Geometry: see drawing. Coordinates: mm, zero at the bounding-box minimum. A direction names the side the tool comes from. Give positions to 0.01 mm unless a question says otherwise; leave off trailing zeros. Loops run counter-clockwise (first coordinate to the right, second up) from the corner with the lowest first, then second, coordinate; pieces in that order, holes last. Notation, with made-up numbers: (39.5, 75) -> (77.5, 75) arc R30 cw to (77.5, 110) -> close; hole circle Ø3 at (-19.75, -7). An arc over 180 degrees is marked (long way). Answer in a Markdown table with one row per item. Add a question column.
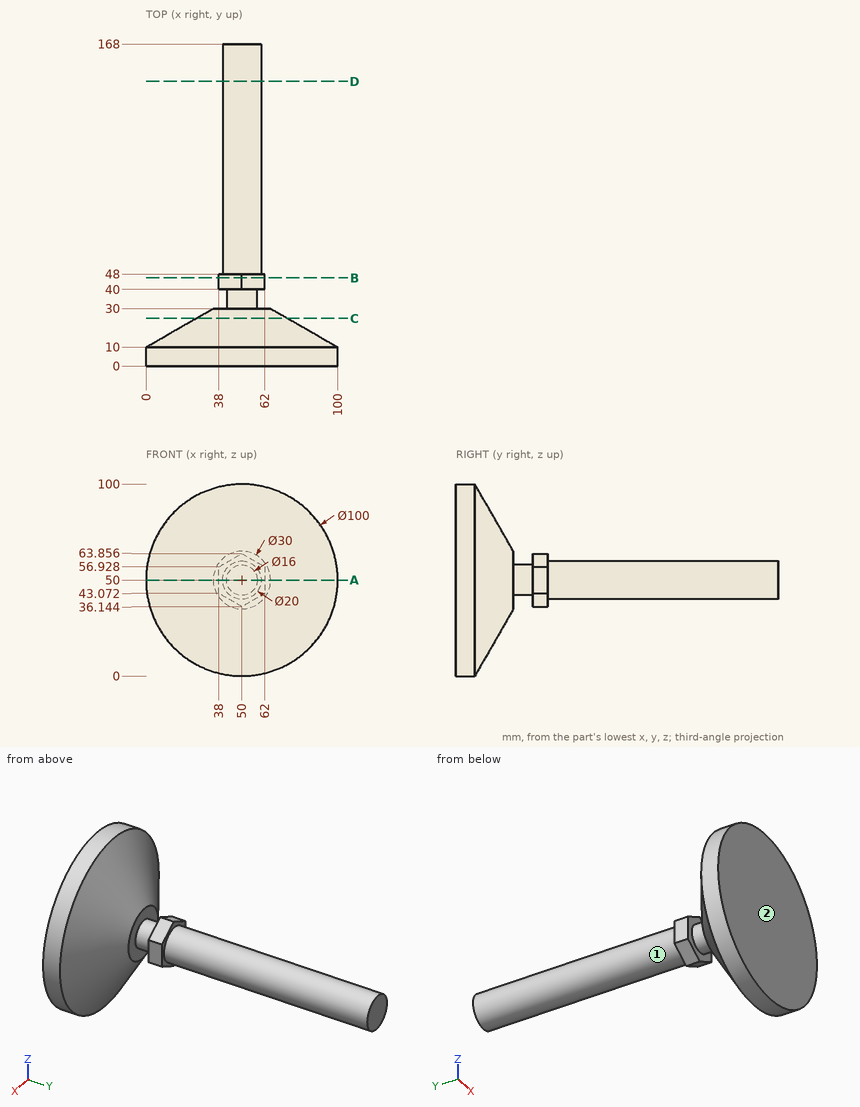
1) Section B-B on y = 46. Output: boundary loops of the cut face in (x, z), and give its area (3 significant figures).
2) Section C-C on y = 25. Output: boundary loops of the cut face in (x, z).
3) Section D-D on y = 148.5. Output: boundary loops of the cut face in (x, z).
4) Reachability of the marked faces 1 and 2 from +Z, -Z, +X, -X, +Y, -Y: full face, straight path, thin tool, end or side. Return the list, or none.
5) Section A-A on z = 50. Output: boundary loops of the cut face in (x, y).
6) Material intervals for line 1 along X through (y, z) = (21, 69) (1 decimal); line 2 along Y through (x, z) = (33, 47); line 3 along Y through (x, z) = (66, 66), sorted ascending.
7) Pin query (flat end, axial travel): pin 1 (12 mm diameter, centred on y = 61.5, z = 41.5, fed in from -X); pin 2 (6 mm diameter, centred on y = 131.5, z = 42, fed in from -X); pin 3 (6.5 mm diameter, centred on y = 42.5, z = 48, fed in from +X); pin 4 (1 mm diameter, centred on x = 38.5, y = 130, fed in from +Z). Return the tip coordinate at first contact, or that it passes through.
Working result:
| question | item | result |
|---|---|---|
| 1 | outline | (38, 43.07) -> (50, 36.14) -> (62, 43.07) -> (62, 56.93) -> (50, 63.86) -> (38, 56.93) -> close |
| 1 | area | 499 mm2 |
| 2 | outline | circle Ø47.5 at (50, 50) |
| 3 | outline | circle Ø20 at (50, 50) |
| 4 | face 1 | +Y |
| 4 | face 2 | +Z, -Z, +X, -X, -Y |
| 5 | outline | (0, 0) -> (100, 0) -> (100, 10) -> (65, 30) -> (58, 30) -> (58, 40) -> (62, 40) -> (62, 48) -> (60, 48) -> (60, 168) -> (40, 168) -> (40, 48) -> (38, 48) -> (38, 40) -> (42, 40) -> (42, 30) -> (35, 30) -> (0, 10) -> close |
| 6 | line 1 | x = 25.8 to 74.2 |
| 6 | line 2 | y = 0 to 28.71 |
| 6 | line 3 | y = 0 to 25.64 |
| 7 | pin 1 | stops at x = 40.32 |
| 7 | pin 2 | stops at x = 41.34 |
| 7 | pin 3 | stops at x = 62 |
| 7 | pin 4 | passes through |
